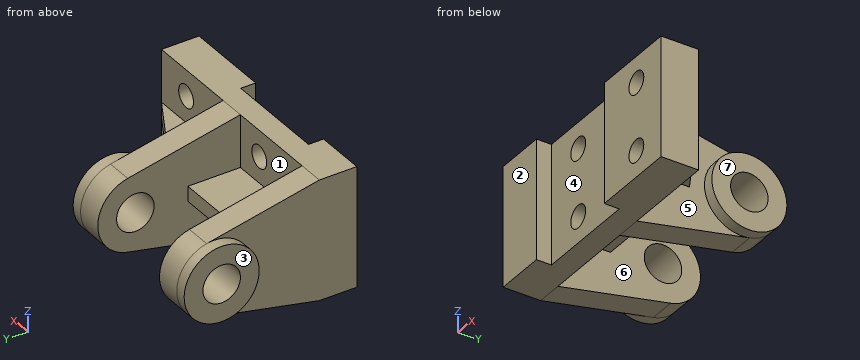
from build123d import *

# Parameters (mm, degrees)
BASE_PLATE_DEPTH        = 64
CLEVIS_LUG_1_DEPTH      = 14
LUG_START               = 6
LUG_1_HUB_SKETCH_R      = 20
LUG_1_HUB_BOSS_40_DEPTH = 6
LUG_1_PIN_BORE_SKETCH_R = 10
LUG_1_PIN_BORE_20_DEPTH = 30
WEB_BLOCK_SKETCH_W      = 50
WEB_BLOCK_SKETCH_H      = 28
WEB_BLOCK_DEPTH         = 64
WEB_TRIM_CUT_1_SKETCH_W = 50
WEB_TRIM_CUT_1_SKETCH_H = 28
WEB_TRIM_CUT_1_DEPTH    = 28
WEB_TRIM_CUT_2_SKETCH_W = 50
WEB_TRIM_CUT_2_SKETCH_H = 28
WEB_TRIM_CUT_2_DEPTH    = 28
CLEVIS_LUG_2_DEPTH      = 14
LUG_2_HUB_SKETCH_R      = 20
LUG_2_HUB_BOSS_40_DEPTH = 6
LUG_START_2             = -30
LUG_2_PIN_BORE_SKETCH_R = 10
LUG_2_PIN_BORE_20_DEPTH = 30
GUSSET_BLOCK_DEPTH      = 64
GUSSET_TRIM_CUT_1_DEPTH = 28
GUSSET_TRIM_CUT_2_DEPTH = 28
MOUNTING_HOLES_SKETCH_R = 6
MOUNTING_HOLES_12_DEPTH = 28


with BuildPart() as part:
    # Base Plate Profile Sketch → Base Plate (new body)
    with BuildSketch(Plane.XY):
        Polygon((0, 0), (27, 0), (82, 0), (128, 0), (128, -20), (82, -20), (82, -12), (27, -12), (27, -20), (0, -20), align=None)
    extrude(amount=-BASE_PLATE_DEPTH)

    # Clevis Lug 1 Sketch → Clevis Lug 1 (add)
    with BuildSketch(Plane.ZY):
        with BuildLine():
            Line((-51.585841233, 60.049052133), (-64, 0))
            Line((-64, 0), (-32, 0))
            Line((-32, 0), (0, 0))
            Line((0, 0), (-12.414158767, 60.049052133))
            ThreePointArc((-12.414158767, 60.049052133), (-32, 76), (-51.585841233, 60.049052133))
        make_face()
    extrude(amount=-CLEVIS_LUG_1_DEPTH)

    # Lug 1 Hub Sketch → Lug 1 Hub Boss Ø40 (add)
    with BuildSketch(Plane.ZY.offset(LUG_START)):
        with Locations((-32, 56)):
            Circle(LUG_1_HUB_SKETCH_R)
    extrude(amount=-LUG_1_HUB_BOSS_40_DEPTH)

    # Lug 1 Pin Bore Sketch → Lug 1 Pin Bore Ø20 (cut)
    with BuildSketch(Plane.ZY.offset(6)):
        with Locations((-32, 56)):
            Circle(LUG_1_PIN_BORE_SKETCH_R)
    extrude(amount=-LUG_1_PIN_BORE_20_DEPTH, mode=Mode.SUBTRACT)

    # Web Block Sketch → Web Block (add)
    with BuildSketch(Plane.XY):
        with Locations((39, 14)):
            Rectangle(WEB_BLOCK_SKETCH_W, WEB_BLOCK_SKETCH_H)
    extrude(amount=-WEB_BLOCK_DEPTH)

    # Web Trim Cut 1 Sketch → Web Trim Cut 1 (cut)
    with BuildSketch(Plane.XY):
        with Locations((39, 14)):
            Rectangle(WEB_TRIM_CUT_1_SKETCH_W, WEB_TRIM_CUT_1_SKETCH_H)
    extrude(amount=-WEB_TRIM_CUT_1_DEPTH, mode=Mode.SUBTRACT)

    # Web Trim Cut 2 Sketch → Web Trim Cut 2 (cut)
    with BuildSketch(Plane(origin=(0, 0, -64), x_dir=(-1, 0, 0), z_dir=(0, 0, -1))):
        with Locations((-39, 14)):
            Rectangle(WEB_TRIM_CUT_2_SKETCH_W, WEB_TRIM_CUT_2_SKETCH_H)
    extrude(amount=-WEB_TRIM_CUT_2_DEPTH, mode=Mode.SUBTRACT)

    # Clevis Lug 2 Sketch → Clevis Lug 2 (add)
    with BuildSketch(Plane(origin=(64, 0, 0), x_dir=(0, 0, -1), z_dir=(1, 0, 0))):
        with BuildLine():
            Line((0, 0), (12.414158767, 60.049052133))
            ThreePointArc((12.414158767, 60.049052133), (32, 76), (51.585841233, 60.049052133))
            Line((51.585841233, 60.049052133), (64, 0))
            Line((64, 0), (0, 0))
        make_face()
    extrude(amount=CLEVIS_LUG_2_DEPTH)

    # Lug 2 Hub Sketch → Lug 2 Hub Boss Ø40 (add)
    with BuildSketch(Plane(origin=(78, 0, 0), x_dir=(0, 0, -1), z_dir=(1, 0, 0))):
        with Locations(Location((32, 56, 0), (0, 0, 180))):
            Circle(LUG_2_HUB_SKETCH_R)
    extrude(amount=LUG_2_HUB_BOSS_40_DEPTH)

    # Lug 2 Pin Bore Sketch → Lug 2 Pin Bore Ø20 (cut)
    with BuildSketch(Plane(origin=(84, 0, 0), x_dir=(0, 0, -1), z_dir=(1, 0, 0)).offset(LUG_START_2)):
        with Locations(Location((32, 56, 0), (0, 0, 180))):
            Circle(LUG_2_PIN_BORE_SKETCH_R)
    extrude(amount=LUG_2_PIN_BORE_20_DEPTH, mode=Mode.SUBTRACT)

    # Gusset Block Sketch → Gusset Block (add)
    with BuildSketch(Plane.XY):
        Polygon((78, 0), (78, 28), (128, 0), align=None)
    extrude(amount=-GUSSET_BLOCK_DEPTH)

    # Gusset Trim Cut 1 Sketch → Gusset Trim Cut 1 (cut)
    with BuildSketch(Plane.XY):
        Polygon((78, 28), (78, 0), (128, 0), align=None)
    extrude(amount=-GUSSET_TRIM_CUT_1_DEPTH, mode=Mode.SUBTRACT)

    # Gusset Trim Cut 2 Sketch → Gusset Trim Cut 2 (cut)
    with BuildSketch(Plane(origin=(0, 0, -64), x_dir=(-1, 0, 0), z_dir=(0, 0, -1))):
        Polygon((-128, 0), (-78, 0), (-78, 28), align=None)
    extrude(amount=-GUSSET_TRIM_CUT_2_DEPTH, mode=Mode.SUBTRACT)

    # Mounting Holes Sketch → Mounting Holes Ø12 (cut)
    with BuildSketch(Plane(origin=(0, 0, 0), x_dir=(1, 0, 0), z_dir=(0, 1, 0))):
        with Locations(Location((48.7, 50, 0), (0, 0, 270))):
            Circle(MOUNTING_HOLES_SKETCH_R)
        with Locations(Location((108, 50, 0), (0, 0, 270))):
            Circle(MOUNTING_HOLES_SKETCH_R)
        with Locations(Location((108, 14, 0), (0, 0, 270))):
            Circle(MOUNTING_HOLES_SKETCH_R)
        with Locations(Location((48.7, 14, 0), (0, 0, 270))):
            Circle(MOUNTING_HOLES_SKETCH_R)
    extrude(amount=-MOUNTING_HOLES_12_DEPTH, mode=Mode.SUBTRACT)


solid = part.part
Input: part model. Units: mm. Frame: model coordinates. Face numbers are marked on the shaded views. A direction names the side the tool comes from. Give positions to 0.01 mm unless a question says otherwise; leave off trailing zeros. Order: outer loops, then holes, each group sorted by start corner. A loop starts at its lowest first (then second) coordinate and runs counter-clockwise, first axis right, second up. Notation, with made-up numbers: (24, 47) - (72, 47) arc R28 cw to (72, 81) - close; hole circle Ø4 at (-23.75, 46.25). An arc over 180 degrees is marked (long way). Write each question's results on one line, items separated by ' | '.
Item 1: Section D-D (x = 9.5). Return loops of the section in (y, z).
A:
outline: (-20, -64) - (0, -64) - (60.05, -51.59) arc R20 ccw to (60.05, -12.41) - (0, 0) - (-20, 0) - close; hole circle Ø20 at (56, -32)
Item 2: Contact query for flat-ended pins moving along their axis: pin 1 Ø9.5 at (x, z) = (48.7, -14) entering from +Y (3 decimals); pin 2 Ø9 at (y, z) = (-16, -18) entering from -X; pin 3 Ø12 at (x, y) = (88.5, 14) entering from +Z; pin 4 Ø8 at (x, z) = (65.5, -22) entering from +Y. Output: stop coordinate, or through.
A:
pin 1: passes through | pin 2: stops at x = 0 | pin 3: stops at z = -28 | pin 4: stops at y = 75.08
Item 3: Material intervals for line 1 along X through (y, z) = (-4, -50); line 2 along X through (y, z) = (8.5, -17); line 3 along Y through (x, z) = (79, -35), sorted ascending.
A:
line 1: x = 0 to 42.7, 54.7 to 102, 114 to 128 | line 2: x = 0 to 14, 64 to 78 | line 3: y = -12 to 27.44, 36.23 to 46.46, 65.54 to 75.77
Item 4: Section C-C (y = -8). Return loops of the section in (x, z).
A:
outline: (0, -64) - (128, -64) - (128, 0) - (0, 0) - close; hole circle Ø12 at (48.7, -50); hole circle Ø12 at (48.7, -14); hole circle Ø12 at (108, -50); hole circle Ø12 at (108, -14)
Item 5: Section A-A (x = 108). Return loops of the section in (y, z), and give its area (3 significant figures).
A:
outline: (-20, -64) - (0, -64) - (0, -56) - (-20, -56) - close; (-20, -44) - (0, -44) - (0, -36) - (11.2, -36) - (11.2, -28) - (0, -28) - (0, -20) - (-20, -20) - close; (-20, -8) - (0, -8) - (0, 0) - (-20, 0) - close | area: 890 mm^2
Item 6: Access query for the marked faces 4, 5, 6 and 7. Directions: +Z, -Z, +X, -X, +Y, -Y. A direction counts if a zero-diameter tool reaches every point of the face in a straight line with its end or side. Return the directions, or none.
A:
face 4: +Z, -Z, -Y | face 5: +X | face 6: +Y | face 7: +Z, -Z, +X, +Y
Item 7: Section B-B (z = -32). Return loops of the section in (x, y), and give its area (3 significant figures).
A:
outline: (-6, 36) - (0, 36) - (0, -20) - (27, -20) - (27, -12) - (82, -12) - (82, -20) - (128, -20) - (128, 0) - (78, 28) - (78, 36) - (84, 36) - (84, 46) - (64, 46) - (64, 28) - (14, 28) - (14, 46) - (-6, 46) - close; (-6, 66) - (14, 66) - (14, 76) - (-6, 76) - close; (64, 66) - (84, 66) - (84, 76) - (64, 76) - close | area: 6,030 mm^2
Item 8: Draft query along X for the marked faces 1, 2 and 3. Return one class per face: released by +X, released by -X, zero draft, split by the parting line, or undercut.
A:
face 1: undercut | face 2: zero draft | face 3: released by -X
